Could you check a few things on this drawing? It's one solid part, dimensions in mm from its lowest x, y, z. A direction names the side the tool comes from. Round coordinates to 2 decimals unless told otherwise and drop trailing zeros. Loops run counter-clockwise (first coordinate to the right, second up) from the corner with the lowest first, then second, coordinate; pieces in that order, holes last. Notation, with made-up numbers: M 55,86.5 L 61,86.5 A37 ccw 61,125.5 Z; hole C 66,76.5 d8. An arc over 180 degrees is marked long. Write each question's results on one line, items separated by ' | '. Start each with the question number.
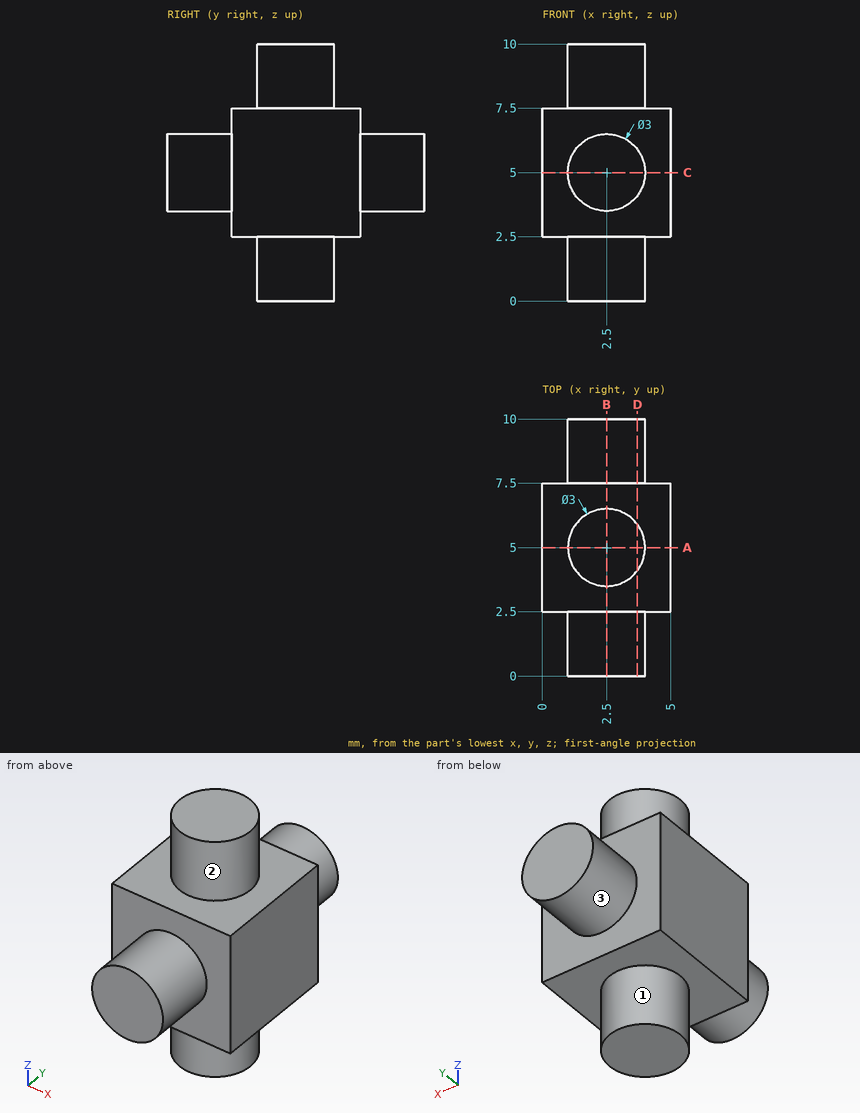
1. I need wall thicknesses on line 1 along Y through (x, z) = (4, 6); line 2 along Y through (x, z) = (2.5, 9.75). Which ranges of each line are inside material? Lowest first, please.
2. I want a section at B-B on x = 2.5. List the corners of the cut face in (y, z) for me.
3. I want a section at A-A on y = 5. List the corners of the cut face in (x, z) for me, plus the area to 3 significant figures.
4. For pin 1 (1.5 mm diameter, centred on x = 1.5, y = 7.5, fed in from -Z), with a flat end and sliding along its axis, tell me the tip position at first contact or that it passes through.
5. Which directions (+Z, -Z, +X, -X, +Y, -Y) give clear straight access to the entire face, cutting with the end or side of a thin tool? Please do the marked faces 1, 2 and 3.
6. I want a section at D-D on x = 3.7. List the corners of the cut face in (y, z) for me.
Outcome:
1) line 1: 2.5 to 7.5 | line 2: 3.5 to 6.5
2) outline: M 0,3.5 L 2.5,3.5 L 2.5,2.5 L 3.5,2.5 L 3.5,0 L 6.5,0 L 6.5,2.5 L 7.5,2.5 L 7.5,3.5 L 10,3.5 L 10,6.5 L 7.5,6.5 L 7.5,7.5 L 6.5,7.5 L 6.5,10 L 3.5,10 L 3.5,7.5 L 2.5,7.5 L 2.5,6.5 L 0,6.5 Z
3) outline: M 0,2.5 L 1,2.5 L 1,0 L 4,0 L 4,2.5 L 5,2.5 L 5,7.5 L 4,7.5 L 4,10 L 1,10 L 1,7.5 L 0,7.5 Z | area: 40.0 mm2
4) pin 1: z = 2.5
5) face 1: -Z | face 2: +Z | face 3: +Y
6) outline: M 0,4.1 L 2.5,4.1 L 2.5,2.5 L 4.1,2.5 L 4.1,0 L 5.9,0 L 5.9,2.5 L 7.5,2.5 L 7.5,4.1 L 10,4.1 L 10,5.9 L 7.5,5.9 L 7.5,7.5 L 5.9,7.5 L 5.9,10 L 4.1,10 L 4.1,7.5 L 2.5,7.5 L 2.5,5.9 L 0,5.9 Z
